from build123d import *

# Parameters (mm, degrees)
SKETCH1_R           = 98
SKETCH1_R_2         = 63
BOSS_EXTRUDE1_DEPTH = 2
SKETCH2_R           = 94
SKETCH2_R_2         = 65
CUT_EXTRUDE2_DEPTH  = 5
BOSS_EXTRUDE2_DEPTH = 2
BOSS_EXTRUDE7_DEPTH = 2
BOSS_EXTRUDE9_DEPTH = 2
FILLET1_R           = 1


with BuildPart() as part:
    # Sketch1 → Boss-Extrude1 (new body)
    with BuildSketch(Plane.XY):
        Circle(SKETCH1_R)
        Circle(SKETCH1_R_2, mode=Mode.SUBTRACT)
    extrude(amount=BOSS_EXTRUDE1_DEPTH)

    # Sketch2 → Cut-Extrude2 (cut)
    with BuildSketch(Plane.XY.offset(2)):
        Circle(SKETCH2_R)
        Circle(SKETCH2_R_2, mode=Mode.SUBTRACT)
    extrude(amount=-CUT_EXTRUDE2_DEPTH, mode=Mode.SUBTRACT)


with BuildPart() as cut_extrude2_piece_1:
    # of the separate pieces the step leaves, piece 1, a body of its own (cut_extrude2_pieces)
    add(part.part.solids().sort_by_distance((98, 0, 0))[0])



with BuildPart() as cut_extrude2_piece_2:
    # of the separate pieces the step leaves, piece 2, a body of its own (cut_extrude2_pieces)
    add(part.part.solids().sort_by_distance((65, 0, 0))[0])


with BuildPart() as cut_extrude2_piece_1_1:
    add(cut_extrude2_piece_1.part)

    add(cut_extrude2_piece_2.part)  # Boss-Extrude2 merges Cut-Extrude2 piece 2
    # Sketch3 → Boss-Extrude2 (add)
    with BuildSketch(Plane.XY.offset(2)):
        with BuildLine():
            Line((4.836242993, 93.875506676), (4.076760177, 64.872028074))
            ThreePointArc((4.076760177, 64.872028074), (0, 65), (-4.076760177, 64.872028074))
            Line((-4.076760177, 64.872028074), (-4.836242993, 93.875506676))
            ThreePointArc((-4.836242993, 93.875506676), (0, 94), (4.836242993, 93.875506676))
        make_face()
        with BuildLine():
            Line((75.121929416, 56.503944294), (51.501653321, 39.655765094))
            ThreePointArc((51.501653321, 39.655765094), (53.887442216, 36.347538726), (56.061044042, 32.896190372))
            Line((56.061044042, 32.896190372), (80.530714938, 48.485089992))
            ThreePointArc((80.530714938, 48.485089992), (77.92953182, 52.564132926), (75.121929416, 56.503944294))
        make_face()
        with BuildLine():
            Line((-93.289131575, 11.538541067), (-64.594398177, 7.250084427))
            ThreePointArc((-64.594398177, 7.250084427), (-64.012503946, 11.287131548), (-63.178554226, 15.279734486))
            Line((-63.178554226, 15.279734486), (-91.60952201, 21.064080257))
            ThreePointArc((-91.60952201, 21.064080257), (-92.571928783, 16.322928701), (-93.289131575, 11.538541067))
        make_face()
    extrude(amount=-BOSS_EXTRUDE2_DEPTH)

    # Sketch8 → Boss-Extrude7 (add)
    with BuildSketch(Plane.XY.offset(2)):
        with BuildLine():
            Line((-52.42405813, -38.428090366), (-79.6500328, -49.918656582))
            ThreePointArc((-79.6500328, -49.918656582), (0, -94), (79.6500328, -49.918656582))
            Line((79.6500328, -49.918656582), (52.42405813, -38.428090366))
            ThreePointArc((52.42405813, -38.428090366), (0, -65), (-52.42405813, -38.428090366))
        make_face()
    extrude(amount=-BOSS_EXTRUDE7_DEPTH)

    # Sketch9 → Boss-Extrude9 (add, symmetric)
    with BuildSketch(Plane.XY.offset(2)):
        with BuildLine():
            Line((68.281233408, -34.472640013), (63.286378857, -43.012470433))
            Line((63.286378857, -43.012470433), (79.6500328, -49.918656582))
            ThreePointArc((79.6500328, -49.918656582), (82.146531581, -45.694062516), (84.419166177, -41.344943851))
            Line((84.419166177, -41.344943851), (69.584267033, -34.079436503))
            ThreePointArc((69.584267033, -34.079436503), (68.855533807, -34.020151468), (68.281233408, -34.472640013))
        make_face()
        with BuildLine():
            Line((67.88695627, -33.166048499), (62.357246072, -42.620335278))
            Line((62.357246072, -42.620335278), (63.286378857, -43.012470433))
            Line((63.286378857, -43.012470433), (68.281233408, -34.472640013))
            ThreePointArc((68.281233408, -34.472640013), (68.855533807, -34.020151468), (69.584267033, -34.079436503))
            Line((69.584267033, -34.079436503), (84.419166177, -41.344943851))
            ThreePointArc((84.419166177, -41.344943851), (84.63789491, -40.895314466), (84.854228869, -40.444527975))
            Line((84.854228869, -40.444527975), (69.189989894, -32.772844989))
            ThreePointArc((69.189989894, -32.772844989), (68.461256668, -32.713559953), (67.88695627, -33.166048499))
        make_face()
        with BuildLine():
            Line((62.357246072, -42.620335278), (57.396762094, -51.10140145))
            ThreePointArc((57.396762094, -51.10140145), (49.408790851, -52.744247062), (48.625615223, -44.626780572))
            ThreePointArc((48.625615223, -44.626780572), (51.08046785, -41.794566683), (53.370590226, -38.8275688))
            Line((53.370590226, -38.8275688), (52.42405813, -38.428090366))
            ThreePointArc((52.42405813, -38.428090366), (50.232411211, -41.251725587), (47.888863477, -43.95061723))
            ThreePointArc((47.888863477, -43.95061723), (48.814898229, -53.548791376), (58.259955891, -51.606274177))
            Line((58.259955891, -51.606274177), (63.286378857, -43.012470433))
            Line((63.286378857, -43.012470433), (62.357246072, -42.620335278))
        make_face()
    extrude(amount=BOSS_EXTRUDE9_DEPTH, both=True)

    # Fillet1
    fillet1_edges = [cut_extrude2_piece_1_1.edges().sort_by_distance(p)[0] for p in [
        (63.286378857, -43.012470433, 3),
    ]]
    fillet(fillet1_edges, radius=FILLET1_R)


solid = cut_extrude2_piece_1_1.part
Geometry check sheet. Reference: the model listing, model coordinates, mm. A direction names the side the tool comes from. Give positions to 0.01 mm unless a question says otherwise; leave off trailing zeros. Write each loop counter-clockwise with the first axis right and the second up, starting at its lowest first coordinate (ties: lowest second). Pieces come first, ordered by that corner, then holes.
1) Cross-section at B-B (x = 0). Record the boundary of the cut face in (y, z).
Values follow:
outline: (-98, 0) - (-63, 0) - (-63, 2) - (-98, 2) - close; (63, 0) - (98, 0) - (98, 2) - (63, 2) - close
2) Cross-section at D-D (x = -67.5). Record the boundary of the cut face in (y, z).
Values follow:
outline: (-71.05, 0) - (-44.79, 0) - (-44.79, 2) - (-71.05, 2) - close; (7.68, 0) - (16.16, 0) - (16.16, 2) - (7.68, 2) - close; (65.42, 0) - (71.05, 0) - (71.05, 2) - (65.42, 2) - close
3) Cross-section at A-A (y = 0). Record the boundary of the cut face in (x, z), plus the area to 3 significant figures.
Values follow:
outline: (-98, 0) - (-94, 0) - (-94, 2) - (-98, 2) - close; (-65, 0) - (-63, 0) - (-63, 2) - (-65, 2) - close; (63, 0) - (65, 0) - (65, 2) - (63, 2) - close; (94, 0) - (98, 0) - (98, 2) - (94, 2) - close
area: 24.0 mm2
4) Thickness scan on line 1 (X direction, y = -24.5, z = 0.7); line 2 (X direction, y = 67, z = 1.9); line 3 (Y direction, x = 21, z = 1.2). Record the ranges inside material, lowest first.
Values follow:
line 1: x = -94.89 to -90.75, -60.21 to -58.04, 58.04 to 60.21, 90.75 to 94.89
line 2: x = -71.52 to -65.93, -4.13 to 4.13, 65.93 to 71.52
line 3: y = -95.72 to -59.4, 59.4 to 61.51, 91.62 to 95.72
5) Cross-section at C-C (z = 0.65). Record the boundary of the cut face in (x, y).
Values follow:
outline: circle Ø196 at (0, 0); hole (-93.29, 11.54) arc R94 ccw to (-79.65, -49.92) - (-52.42, -38.43) arc R65 cw to (-64.59, 7.25) - close; hole (-91.61, 21.06) - (-63.18, 15.28) arc R65 cw to (-4.08, 64.87) - (-4.84, 93.88) arc R94 ccw to start; hole circle Ø126 at (0, 0); hole (4.08, 64.87) arc R65 cw to (51.5, 39.66) - (75.12, 56.5) arc R94 ccw to (4.84, 93.88) - close; hole (52.42, -38.43) - (62.36, -42.62) - (67.89, -33.17) arc R1 cw to (69.19, -32.77) - (84.85, -40.44) arc R94 ccw to (80.53, 48.49) - (56.06, 32.9) arc R65 cw to start
6) Set-up check for faces 4 (the face through (70, -42, 4)), 5 (the face through (71.76, -46.59, 3.01)), 6 (the face through (-59.77, 72.55, 1.01)), 7 (the face through (49.513, -52.819, 3.014)): record each of +Z, -Z, +X, -X, +Y, -Y from which the full face is reachable in a straight line by a thin tool's end or side.
Values follow:
face 4: +Z, +X, -X, +Y, -Y
face 5: +Z, -Y
face 6: +Z, -Z
face 7: +Z
7) Release check for a two-part mould opening along X. For faces 1 (the face through (-8.201, 62.464, 0.986)), 2 (the face through (7, -65, 0)), 3 (the face through (52.684, 82.634, 0.986)) record: released by +X, released by -X, zero draft, split by the parting line, or undercut.
Values follow:
face 1: undercut
face 2: zero draft
face 3: split by the parting line
